Verification items for the finished model (mm, model axes). A direction names the side the tool comes from. Round coordinates to 2 decimals unless told otherwise and drop trailing zeros. Order: outer loops, then holes, each group sorted by start corner. A loop starts at its lowest first (then second) coordinate and runs counter-clockwise, first axis right, second up. Notation, with made-up numbers: M -27,-21.75 L -16,-21.75 A32 ccw -16,10.25 Z; hole C 72,26 d4. An arc over 180 degrees is marked long. Use CSV: the item, a comma, the result in double quotes. Start each with the question number.
Q1. Mould release check, pull along X, two halves, no side actions. Record for faces 4 (the face through (27.146, 5.423, 8.176)), 5 (the face through (70, 8, 7)), 6 (the face through (8, 36, 7)): +X half, -X half, draft (parallel to the pull), parting line (faces both ways), or undercut.
Q2. Sectioned sample at A-A (z = 7.5). Enter the section's corners in (x, y), and give its area (3 significant figures).
Q3. Set-up check for faces 1 (the face through (27, 10, 15)), 2 (the face through (65.994, 13.535, 7.764)), 3 (the face through (15, 23, 7)): record each of +Z, -Z, +X, -X, +Y, -Y from which the full face is reachable in a straight line by a thin tool's end or side.
Q4. Gauge pin test, flat ends, axial feed: pin 1 Ø1.5 at (x, z) = (54.5, 11) entering from -Y; pin 2 Ø6 at (x, z) = (25.5, 6.5) entering from +Y; pin 3 Ø3.5 at (x, z) = (60, 7.5) entering from -Y. Record the tip position at first contact, or that the pin passes through.
Q5. Scan lines: line 1 (Z direction, x = 25, y = 4); line 2 (Z direction, x = 60, y = 12.3); line 3 (Y direction, x = 26, z = 2.5). Record each from-to range of solid material in increasing order.
Q6. Sectioned sample at C-C (y = 7.5). Enter the section's corners in (x, z).
Q7. Sectioned sample at D-D (x = 51). Enter the section's corners in (y, z).
Q8. Sectioned sample at B-B (x = 25). Enter the section's corners in (y, z), and give its area (4 significant figures).
```python
from build123d import *

# Parameters (mm, degrees)
EXTRUDE_1_DEPTH           = 15
FILLET_1_R                = 5
HOLE_WIZARD_1_D           = 4.5
HOLE_WIZARD_1_DEPTH       = 100
HOLE_WIZARD_1_CBORE_D     = 12
HOLE_WIZARD_1_CBORE_DEPTH = 5


with BuildPart() as part:
    # 草图1 → 凸台-拉伸1 (new body)
    with BuildSketch(Plane.XY):
        Polygon((0, 0), (70, 0), (70, 16), (15, 16), (15, 36), (0, 36), (0, 16), align=None)
    extrude(amount=EXTRUDE_1_DEPTH)

    # 圆角1
    fillet_1_edges = [part.edges().sort_by_distance(p)[0] for p in [
        (0, 36, 7.5),
        (15, 36, 7.5),
    ]]
    fillet(fillet_1_edges, radius=FILLET_1_R)

    # 孔1
    with Locations(Plane(origin=(0, 16, 0), x_dir=(-1, 0, 0), z_dir=(0, 1, 0))):
        with Locations((-25, 7.5), (-60, 7.5)):
            CounterBoreHole(HOLE_WIZARD_1_D / 2, HOLE_WIZARD_1_CBORE_D / 2, HOLE_WIZARD_1_CBORE_DEPTH, depth=HOLE_WIZARD_1_DEPTH)


solid = part.part
```
Verdict:
1,face 4,"undercut"
1,face 5,"+X half"
1,face 6,"draft"
2,outline,"M 0,0 L 22.75,0 L 22.75,11 L 19,11 L 19,16 L 15,16 L 15,31 A5 ccw 10,36 L 5,36 A5 ccw 0,31 Z; M 27.25,0 L 57.75,0 L 57.75,11 L 54,11 L 54,16 L 31,16 L 31,11 L 27.25,11 Z; M 62.25,0 L 70,0 L 70,16 L 66,16 L 66,11 L 62.25,11 Z"
2,area,"1,190 mm²"
3,face 1,"+Z, +X, -X, +Y, -Y"
3,face 2,"+Y"
3,face 3,"+Z, -Z, +X, +Y"
4,pin 1,"stops at y = 0"
4,pin 2,"stops at y = 11"
4,pin 3,"passes through"
5,line 1,"z = 0 to 5.25, 9.75 to 15"
5,line 2,"z = 0 to 1.5, 13.5 to 15"
5,line 3,"y = 0 to 11"
6,outline,"M 0,0 L 70,0 L 70,15 L 0,15 Z; hole C 25,7.5 d4.5; hole C 60,7.5 d4.5"
7,outline,"M 0,0 L 16,0 L 16,15 L 0,15 Z"
8,outline,"M 0,0 L 16,0 L 16,1.5 L 11,1.5 L 11,5.25 L 0,5.25 Z; M 0,9.75 L 11,9.75 L 11,13.5 L 16,13.5 L 16,15 L 0,15 Z"
8,area,"130.5 mm²"
